```python
from build123d import *

# Parameters (mm, degrees)
MID_SECTION_PROFILE_W = 33
MID_SECTION_PROFILE_H = 6.5
TIP_DOME_FILLET_R8_R  = 8
END_FLARE_FILLET_R3_R = 3


with BuildPart() as part:
    # Shaft Core Profile → Shaft Core Revolve (revolve)
    with BuildSketch(Plane.XY, mode=Mode.PRIVATE) as shaft_core_revolve_sk:
        Polygon((0, 0), (0, 9), (0.5, 9), (0.5, 9.5), (5, 9.5), (5, 9), (5.5, 9), (5.5, 8.7), (19.5, 7), (19.5, 9), (20, 9), (20, 9.5), (24.5, 9.5), (24.5, 9), (25, 9), (25, 0), align=None)
    revolve(shaft_core_revolve_sk.sketch.rotate(Axis((0, 0, 0), (1, 0, 0)), 90), axis=Axis((0, 0, 0), (1, 0, 0)))

    # Mid Section Profile → Mid Section Revolve (revolve)
    with BuildSketch(Plane.XY, mode=Mode.PRIVATE) as mid_section_revolve_sk:
        with Locations((41.5, 3.25)):
            Rectangle(MID_SECTION_PROFILE_W, MID_SECTION_PROFILE_H)
    revolve(mid_section_revolve_sk.sketch.rotate(Axis((25, 0, 0), (1, 0, 0)), 90), axis=Axis((25, 0, 0), (1, 0, 0)))

    # Collars Profile → Collars Revolve (revolve)
    with BuildSketch(Plane.XY, mode=Mode.PRIVATE) as collars_revolve_sk:
        Polygon((58, 0), (58, 8.5), (59, 8.5), (59, 9.5), (63, 9.5), (63, 8.5), (64, 8.5), (64, 7.25), (86, 7.25), (86, 8.5), (87, 8.5), (87, 9.5), (91, 9.5), (91, 8.5), (92, 8.5), (92, 7.5), (99, 7.5), (99, 8.5), (100, 8.5), (100, 9.5), (104, 9.5), (104, 8.5), (105, 8.5), (105, 8), (120, 8), (128, 8), (128, 0), align=None)
    revolve(collars_revolve_sk.sketch.rotate(Axis((58, 0, 0), (1, 0, 0)), 90), axis=Axis((58, 0, 0), (1, 0, 0)))

    # Tip Dome Fillet R8
    tip_dome_fillet_r8_edges = [part.edges().sort_by_distance(p)[0] for p in [
        (128, 0, -8),
    ]]
    fillet(tip_dome_fillet_r8_edges, radius=TIP_DOME_FILLET_R8_R)

    # End Flare Profile → End Flare Revolve (revolve)
    with BuildSketch(Plane.XY, mode=Mode.PRIVATE) as end_flare_revolve_sk:
        with BuildLine():
            Line((124.926812112, 0), (124.926812112, 3))
            Line((124.926812112, 3), (132.926812112, 3))
            ThreePointArc((132.926812112, 3), (133.926812112, 2), (134.926812112, 3))
            Line((134.926812112, 3), (139.926812112, 3))
            Line((139.926812112, 3), (142.926812112, 3))
            Line((142.926812112, 3), (142.926812112, 0))
            Line((142.926812112, 0), (124.926812112, 0))
        make_face()
    revolve(end_flare_revolve_sk.sketch.rotate(Axis((124.926812112, 0, 0), (1, 0, 0)), 90), axis=Axis((124.926812112, 0, 0), (1, 0, 0)))

    # End Flare Fillet R3
    end_flare_fillet_r3_edges = [part.edges().sort_by_distance(p)[0] for p in [
        (142.926812112, 0, -3),
    ]]
    fillet(end_flare_fillet_r3_edges, radius=END_FLARE_FILLET_R3_R)


solid = part.part
```
Geometry check sheet. Reference: the model listing, model coordinates, mm. A direction names the side the tool comes from. Coordinates: 2 decimals unless noted, no trailing zeros. Order: outer loops, then holes, each group sorted by start corner. A loop starts at its lowest first (then second) coordinate and runs counter-clockwise, first axis right, second up. Notation, with made-up numbers: M -25,42 L 33,42 A19 cw 33,55 Z; hole C -3.5,-33 d5. An arc over 180 degrees is marked long. One line per question, with ' | ' between items. Start each with the question number.
Item 1: Draft check along X on faces 4 (the flat face through (92, 8, 0)), 5 (the cylindrical face through (61.028, 9.274, -2.059)), 6 (the cylindrical face through (24.754, -6.083, -6.633)). Enter one of: pulls with the +X half, pulls with the -X half, needs draft (parallel to the pull), parting line crosses it, or undercut.
Item 2: Gauge pin test, flat ends, axial feed: pin 1 (5 mm diameter, centred on y = 1.5, z = -3, fed in from -X); pin 2 (4 mm diameter, centred on x = 90, y = -6, fed in from +Z); pin 3 (4 mm diameter, centred on x = 102, z = 5, fed in from +Y); pin 4 (3 mm diameter, centred on x = 34.5, y = -6, fed in from +Z). Record the tip position at first contact, or that the pin passes through.
Item 3: Set-up check for faces 1 (the cylindrical face through (91.507, -8.428, -1.107)), 2 (the cylindrical face through (89.028, 9.274, -2.059)), 3 (the cylindrical face through (130.21, -0.9, 2.86)): record each of +Z, -Z, +X, -X, +Y, -Y from which the full face is reachable in a straight line by a thin tool's end or side.
Item 4: Cross-section at A-A on x = 129.5. Enter the section's corners in (y, z), then the cut area to 3 significant figures.
Item 5: Material ranges on L1, parallel to X at y = -3.75, z = -8.25; L2, parallel to Y at x = 101, z = 0; L3, parallel to X at y = 5.75, z = -3.25, recorded low to high. Write a range as [from, to].
Item 6: Cross-section at B-B on x = 66. Enter the section's corners in (y, z), then the cut area to 3 significant figures.
Findings:
1) face 4: undercut | face 5: needs draft | face 6: undercut
2) pin 1: stops at x = 0 | pin 2: stops at z = 8.62 | pin 3: stops at y = 9.01 | pin 4: stops at z = 4.69
3) face 1: none | face 2: +X, -X | face 3: +X
4) outline: C 0,0 d6 | area: 28.3 mm²
5) L1: x = [0.5, 5], [20, 24.5], [59, 63], [87, 91], [100, 104] | L2: y = [-9.5, 9.5] | L3: x = [0, 25], [58, 124.51]
6) outline: C 0,0 d14.5 | area: 165 mm²
